Input: part model. Units: mm. Frame: model coordinates. Face numbers are marked on the shaded views. A direction names the side the tool comes from. Round coordinates to 2 decimals unless told otherwise and drop trailing zeros. Order: outer loops, then holes, each group sorted by start corner. A loop starts at its lowest first (then second) coordinate and runs counter-clockwise, first axis right, second up. Notation, with made-up numbers: (26, 50) -> (72, 50) arc R17 ccw to (72, 67) -> close; hole circle Ø8 at (0.5, -23). An arc over 180 degrees is marked (long way). Use a Markdown table: item, result.
from build123d import *

# Parameters (mm, degrees)
ANGLED_BASE_BLOCK_DEPTH  = 40
GROOVE_CUT_5MM_DEPTH     = 5
T_SLOT_THROUGH_CUT_DEPTH = 40


with BuildPart() as part:
    # Base Profile Sketch → Angled Base Block (new body)
    with BuildSketch(Plane.XY):
        Polygon((0, 0), (60, 0), (60, 30), (45, 30), (20, 8), (0, 8), align=None)
    extrude(amount=ANGLED_BASE_BLOCK_DEPTH)

    # Groove Profile Sketch → Groove Cut 5mm (cut)
    with BuildSketch(Plane.ZY):
        Polygon((20, 8), (10, 8), (10, 0), (30, 0), (30, 8), align=None)
    extrude(amount=-GROOVE_CUT_5MM_DEPTH, mode=Mode.SUBTRACT)

    # T-Slot Profile Sketch → T-Slot Through Cut (cut)
    with BuildSketch(Plane(origin=(60, 0, 0), x_dir=(0, 0, -1), z_dir=(1, 0, 0))):
        Polygon((-20, 30), (-25, 30), (-25, 18), (-35, 18), (-35, 13), (-5, 13), (-5, 18), (-15, 18), (-15, 30), align=None)
    extrude(amount=-T_SLOT_THROUGH_CUT_DEPTH, mode=Mode.SUBTRACT)


solid = part.part
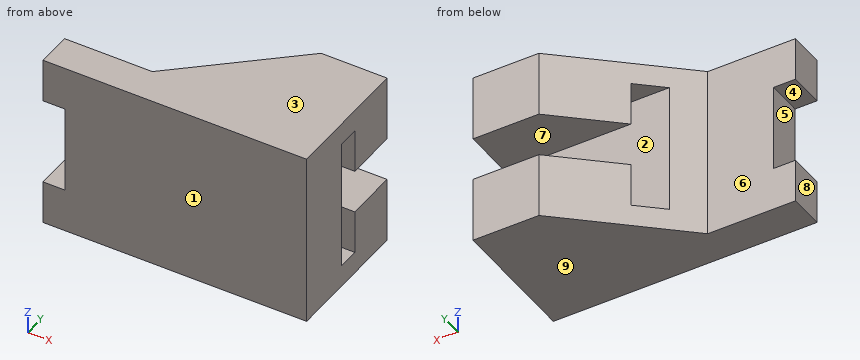
1) Set-up query: the marked faces 5, 6, 7, 8 and 9. Return all of +Z, -Z, +X, -X, +Y, -Y with unobstructed straight access to the full face (end or side cutting, diameter ignored); none if empty.
Answer key:
| item | result |
|---|---|
| face 5 | -X, +Y, -Y |
| face 6 | +Z, -Z, -X, +Y |
| face 7 | +X, -X, +Y |
| face 8 | +Z, -Z, -X, +Y, -Y |
| face 9 | -Z, +X, -X, +Y, -Y |
2) Cut plane A-A on x = 4. Return loops of the section in (y, z), and give its area (3 significant figures).
Answer key:
| item | result |
|---|---|
| outline | (0, 0) -> (8, 0) -> (8, 10) -> (0, 10) -> close; (0, 30) -> (8, 30) -> (8, 40) -> (0, 40) -> close |
| area | 160 mm^2 |
3) Cut plane B-B on z = 33.5. Return loops of the section in (x, y), and give its area (3 significant figures).
Answer key:
| item | result |
|---|---|
| outline | (0, 0) -> (60, 0) -> (60, 13) -> (25.68, 13) -> (20, 8) -> (0, 8) -> close; (31.36, 18) -> (60, 18) -> (60, 30) -> (45, 30) -> close |
| area | 928 mm^2 |
4) Contact query for flat-ended pins moving along their axis: P1, Ø4, axis at x = 20.5, z = 9.5, coming from the +Y side; P2, Ø6.5, axis at y = 3, z = 19.5, coming from the -X side; P3, Ø10, axis at x = 10.5, z = 21, coming from the +Y side. Output: stop coordinate, or through.
Answer key:
| item | result |
|---|---|
| P1 | stops at y = 10.2 |
| P2 | stops at x = 5 |
| P3 | stops at y = 8 |
5) Cut plane D-D on x = 38. Return loops of the section in (y, z), and give its area (3 significant figures).
Answer key:
| item | result |
|---|---|
| outline | (0, 0) -> (23.84, 0) -> (23.84, 15) -> (18, 15) -> (18, 5) -> (13, 5) -> (13, 35) -> (18, 35) -> (18, 25) -> (23.84, 25) -> (23.84, 40) -> (0, 40) -> close |
| area | 745 mm^2 |
6) Ray query, probe 1 along Y at (x, z) = (52, 10); probe 2 along Z at (x, y) = (54.5, 21); probe 3 along Y at (x, z) = (20, 29.5). Return the intervals inside material, ascending.
Answer key:
| item | result |
|---|---|
| probe 1 | y = 0 to 13, 18 to 30 |
| probe 2 | z = 0 to 15, 25 to 40 |
| probe 3 | y = 0 to 8 |
7) Cut plane C-C on y = 14.5. Return loops of the section in (x, z).
Answer key:
| item | result |
|---|---|
| outline | (27.39, 0) -> (60, 0) -> (60, 5) -> (27.39, 5) -> close; (27.39, 35) -> (60, 35) -> (60, 40) -> (27.39, 40) -> close |
8) Draft query along Z for the marked faces 1, 2, 3 and 4. Return one class per face: released by +Z, released by -Z, zero draft, split by the parting line, or undercut.
Answer key:
| item | result |
|---|---|
| face 1 | zero draft |
| face 2 | undercut |
| face 3 | released by +Z |
| face 4 | undercut |
